Here's how the part is built. I have some questions about the finished solid (model axes, mm). Face numbers are marked on the shaded views. A direction names the side the tool comes from. Coordinates: 2 decimals unless noted, no trailing zeros. Order: outer loops, then holes, each group sorted by start corner. A loop starts at its lowest first (then second) coordinate and runs counter-clockwise, first axis right, second up. Notation, with made-up numbers: (40, -10) - (86, -10) arc R12 cw to (86, 11) - close; hole circle Ø4 at (45.5, 14). An arc over 180 degrees is marked (long way). Answer as CSV lines item,"result". Start each with the question number.
Q1. Suppose I cut it at B-B (y = 34.5). Count the separate pieces of the cut face and the enclosed holes in it, then the cut area to 3 significant figures.
Q2. I need wall thicknesses on line 1 (Y direction, x = -34, z = 138); line 2 (Z direction, x = -99, y = 34); line 3 (Z direction, x = -96, y = 46). Which ranges of each line are inside material? Lowest first, please.
Q3. Suppose I cut it at C-C (x = -61). Please give me the cut outline in (y, z), then the cut area to 3 significant figures.
Q4. For the marked faces 1, 2, 3 and 4, which set-ups out of +Z, -Z, +X, -X, +Y, -Y let a thin tool reach every point of the face, with its end or its side?
Q5. Suppose I cut it at A-A (z = 154). Please give me the cut outline in (x, y).
Q6. For pin 1 Ø12 at (y, z) = (40, 132) entering from -X; pin 2 Ø3 at (y, z) = (3.5, 4) entering from -X; pin 3 Ø23 at (x, z) = (-98.17, 149.21) entering from -Y, each with a flat end and sliding along its axis, tell me the tip position at first contact or that it passes through.
Q7. Suppose I cut it at D-D (z = 90). Please give me the cut outline in (x, y), then the cut area to 3 significant figures.
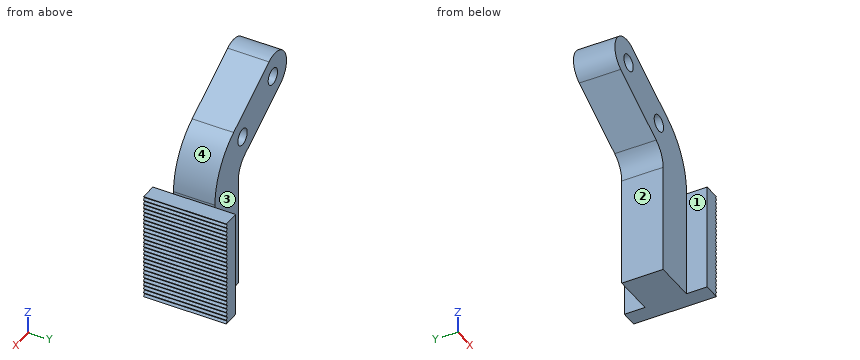
from build123d import *

# Parameters (mm, degrees)
SKETCH1_R           = 10
BOSS_EXTRUDE1_DEPTH = 50
FILLET1_RADIUS      = 25
FILLET1_LENGTH      = 50
SKETCH2_W           = 129.723894377
SKETCH2_H           = 100
BOSS_EXTRUDE2_DEPTH = 20
CUT_EXTRUDE1_DEPTH  = 240.757846963


with BuildPart() as part:
    # Sketch1 → Boss-Extrude1 (new body)
    with BuildSketch(Plane(origin=(0, 0, 0), x_dir=(1, 0, 0), z_dir=(0, 1, 0))):
        with BuildLine():
            Line((-39.067263876, -86.222925476), (-136.650566368, -142.562671438))
            Line((-136.650566368, -142.562671438), (-111.650566368, -185.863941628))
            Line((-111.650566368, -185.863941628), (-14.067263876, -129.524195665))
            ThreePointArc((-14.067263876, -129.524195665), (15.214768427, -100.242163363), (25.932736124, -60.242163363))
            Line((25.932736124, -60.242163363), (25.932736124, 72.437328562))
            Line((25.932736124, 72.437328562), (-24.067263876, 72.437328562))
            Line((-24.067263876, 72.437328562), (-24.067263876, -60.242163363))
            ThreePointArc((-24.067263876, -60.242163363), (-28.086501763, -75.242163363), (-39.067263876, -86.222925476))
        make_face()
        with Locations(Location((-98.169804255, -149.213306533, 0), (0, 0, 270))):
            Circle(SKETCH1_R, mode=Mode.SUBTRACT)
        with Locations(Location((-33.217898971, -111.713306533, 0), (0, 0, 270))):
            Circle(SKETCH1_R, mode=Mode.SUBTRACT)
    extrude(amount=BOSS_EXTRUDE1_DEPTH)

    # Fillet1: full round fillet: the end face becomes a half cylinder, R = half its width
    fillet1_face = Plane((-124.150566368, 25, 164.213306533), x_dir=(0, 1, 0), z_dir=(-0.866025403784, 0, 0.5))  # on the end face: x along it, z out of the body
    fillet1_slab = fillet1_face.offset(-FILLET1_RADIUS / 2) * Box(FILLET1_LENGTH, 2 * FILLET1_RADIUS, FILLET1_RADIUS, mode=Mode.PRIVATE)  # the body's end, R deep
    fillet1_round = Plane((-102.499931273, 25, 151.713306533), x_dir=(-0.866025403784, 0, 0.5), z_dir=(0, 1, 0)) * Cylinder(FILLET1_RADIUS, FILLET1_LENGTH, mode=Mode.PRIVATE)  # its axis R under the face
    add(fillet1_slab - fillet1_round, mode=Mode.SUBTRACT)

    # Sketch2 → Boss-Extrude2 (add)
    with BuildSketch(Plane(origin=(25.932736124, 0, 0), x_dir=(0, 0, -1), z_dir=(1, 0, 0))):
        with Locations((7.575381374, 25)):
            Rectangle(SKETCH2_W, SKETCH2_H)
    extrude(amount=BOSS_EXTRUDE2_DEPTH)

    # Sketch3 → Cut-Extrude1 (cut, through all)
    with BuildSketch(Plane(origin=(0, 75, 0), x_dir=(1, 0, 0), z_dir=(0, 1, 0))):
        Polygon((45.932736124, 67.437328562), (45.932736124, 72.437328562), (43.932736124, 69.937328562), align=None)
        Polygon((45.932736124, 62.437328562), (45.932736124, 67.437328562), (43.932736124, 64.937328562), align=None)
        Polygon((45.932736124, 57.437328562), (45.932736124, 62.437328562), (43.932736124, 59.937328562), align=None)
        Polygon((45.932736124, 52.437328562), (45.932736124, 57.437328562), (43.932736124, 54.937328562), align=None)
        Polygon((45.932736124, 47.437328562), (45.932736124, 52.437328562), (43.932736124, 49.937328562), align=None)
        Polygon((45.932736124, 42.437328562), (45.932736124, 47.437328562), (43.932736124, 44.937328562), align=None)
        Polygon((45.932736124, 37.437328562), (45.932736124, 42.437328562), (43.932736124, 39.937328562), align=None)
        Polygon((45.932736124, 32.437328562), (45.932736124, 37.437328562), (43.932736124, 34.937328562), align=None)
        Polygon((45.932736124, 27.437328562), (45.932736124, 32.437328562), (43.932736124, 29.937328562), align=None)
        Polygon((45.932736124, 22.437328562), (45.932736124, 27.437328562), (43.932736124, 24.937328562), align=None)
        Polygon((45.932736124, 17.437328562), (45.932736124, 22.437328562), (43.932736124, 19.937328562), align=None)
        Polygon((45.932736124, 12.437328562), (45.932736124, 17.437328562), (43.932736124, 14.937328562), align=None)
        Polygon((45.932736124, 7.437328562), (45.932736124, 12.437328562), (43.932736124, 9.937328562), align=None)
        Polygon((45.932736124, 2.437328562), (45.932736124, 7.437328562), (43.932736124, 4.937328562), align=None)
        Polygon((45.932736124, -2.562671438), (45.932736124, 2.437328562), (43.932736124, -0.062671438), align=None)
        Polygon((45.932736124, -7.562671438), (45.932736124, -2.562671438), (43.932736124, -5.062671438), align=None)
        Polygon((45.932736124, -12.562671438), (45.932736124, -7.562671438), (43.932736124, -10.062671438), align=None)
        Polygon((45.932736124, -22.562671438), (45.932736124, -17.562671438), (43.932736124, -20.062671438), align=None)
        Polygon((45.932736124, -27.562671438), (45.932736124, -22.562671438), (43.932736124, -25.062671438), align=None)
        Polygon((45.932736124, -32.562671438), (45.932736124, -27.562671438), (43.932736124, -30.062671438), align=None)
        Polygon((45.932736124, -37.562671438), (45.932736124, -32.562671438), (43.932736124, -35.062671438), align=None)
        Polygon((45.932736124, -42.562671438), (45.932736124, -37.562671438), (43.932736124, -40.062671438), align=None)
        Polygon((45.932736124, -47.562671438), (45.932736124, -42.562671438), (43.932736124, -45.062671438), align=None)
        Polygon((45.932736124, -57.286565815), (45.932736124, -52.562671438), (43.932736124, -55.062671438), (45.711851625, -57.286565815), align=None)
        Polygon((45.932736124, -57.562671438), (45.932736124, -62.562671438), (43.932736124, -60.062671438), align=None)
        Polygon((45.932736124, -12.562671438), (45.932736124, -17.562671438), (43.932736124, -15.062671438), align=None)
        Polygon((45.932736124, -47.562671438), (45.932736124, -52.562671438), (43.932736124, -50.062671438), align=None)
    extrude(amount=-CUT_EXTRUDE1_DEPTH, mode=Mode.SUBTRACT)


solid = part.part
Here are the results:
1,separate pieces,"1"
1,enclosed holes,"2"
1,area,"16,700 mm²"
2,line 1,"y = 0 to 50"
2,line 2,"z = 120.83 to 139.25, 159.18 to 176.47"
2,line 3,"z = 119.09 to 139.45, 158.98 to 175.85"
3,outline,"(0, 98.89) - (50, 98.89) - (50, 156.62) - (0, 156.62) - close"
3,area,"2,890 mm²"
4,face 1,"+Z, -Z, -X, -Y"
4,face 2,"-Z, -X, +Y, -Y"
4,face 3,"+Z, -Z, -X, +Y"
4,face 4,"+Z, +X, +Y, -Y"
5,outline,"(-127.4, 0) - (-106.95, 0) - (-106.95, 50) - (-127.4, 50) - close; (-89.39, 0) - (-56.46, 0) - (-56.46, 50) - (-89.39, 50) - close"
6,pin 1,"stops at x = -123.4"
6,pin 2,"stops at x = -24.07"
6,pin 3,"stops at y = 0"
7,outline,"(-45.61, 0) - (20.19, 0) - (20.19, 50) - (-45.61, 50) - close"
7,area,"3,290 mm²"
